Design review of the part built by this model. Coordinates are the model's own, in mm. Face numbers are marked on the shaded views. A direction names the side the tool comes from. Give positions to 0.01 mm unless a question says otherwise; leave off trailing zeros. Loops run counter-clockwise (first coordinate to the right, second up) from the corner with the lowest first, then second, coordinate; pieces in that order, holes last. Notation, with made-up numbers: (-6.75, 78) - (39.25, 78) arc R30 cw to (39.25, 101) - close; hole circle Ø6 at (31.25, 6.5). An arc over 180 degrees is marked (long way). Write each question's results on one line, items separated by ' | '.
from build123d import *

# Parameters (mm, degrees)
SUPPORT_BLOCK_BODY_DEPTH    = 62
CENTRE_START                = 32
CENTRE_CHANNEL_SKETCH_W     = 60
CENTRE_CHANNEL_SKETCH_H     = 88
CENTRE_CHANNEL_CUT_DEPTH    = 124
V_NOTCH_CUT_DEPTH           = 124
BASE_GROOVE_CUT_18X36_REACH = 97.121
FRONT_NOTCH_CUT_REACH       = 159.899
FRONT_NOTCH_SKETCH_W        = 36
FRONT_NOTCH_SKETCH_H        = 12


with BuildPart() as part:
    # Block Profile Sketch → Support Block Body (new, symmetric)
    with BuildSketch(Plane.XY):
        Polygon((-50, 0), (50, 0), (50, 32), (-10, 84), (-50, 84), align=None)
    extrude(amount=SUPPORT_BLOCK_BODY_DEPTH, both=True)

    # Centre Channel Sketch → Centre Channel Cut (cut)
    with BuildSketch(Plane(origin=(0, 0, 0), x_dir=(1, 0, 0), z_dir=(0, 1, 0)).offset(CENTRE_START)):
        with Locations((20, 0)):
            Rectangle(CENTRE_CHANNEL_SKETCH_W, CENTRE_CHANNEL_SKETCH_H)
    extrude(amount=CENTRE_CHANNEL_CUT_DEPTH, mode=Mode.SUBTRACT)

    # V-Notch Sketch → V-Notch Cut (cut)
    with BuildSketch(Plane(origin=(-10, 0, 0), x_dir=(0, 0, -1), z_dir=(1, 0, 0))):
        Polygon((30, 84), (0, 54), (-30, 84), align=None)
    extrude(amount=-V_NOTCH_CUT_DEPTH, mode=Mode.SUBTRACT)

    # Base Groove Sketch → Base Groove Cut 18x36 (cut, up to next)
    with BuildSketch(Plane(origin=(0, 32, 0), x_dir=(1, 0, 0), z_dir=(0, 1, 0)), mode=Mode.PRIVATE) as base_groove_cut_18x36_sk1:
        Polygon((50, 18), (32, 0), (50, -18), align=None)
    base_groove_cut_18x36_tool1 = extrude(base_groove_cut_18x36_sk1.sketch, amount=-BASE_GROOVE_CUT_18X36_REACH, mode=Mode.PRIVATE) & part.part
    add(base_groove_cut_18x36_tool1.solids().sort_by_distance((44, 32, 0))[0], mode=Mode.SUBTRACT)

    # Front Notch Sketch → Front Notch Cut (cut, up to next)
    with BuildSketch(Plane.XY.offset(62), mode=Mode.PRIVATE) as front_notch_cut_sk1:
        with Locations((0, 6)):
            Rectangle(FRONT_NOTCH_SKETCH_W, FRONT_NOTCH_SKETCH_H)
    front_notch_cut_tool1 = extrude(front_notch_cut_sk1.sketch, amount=-FRONT_NOTCH_CUT_REACH, mode=Mode.PRIVATE) & part.part
    add(front_notch_cut_tool1.solids().sort_by_distance((0, 6, 62))[0], mode=Mode.SUBTRACT)


solid = part.part
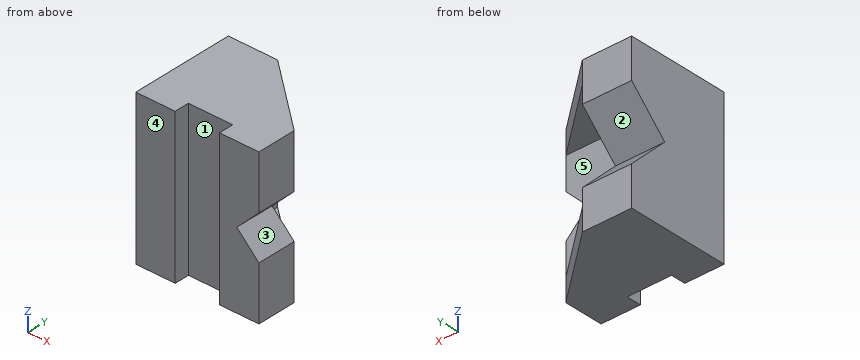
(1) Take a section at D-D on x = -37. Give the boundary of the cut face in (y, z), plus the area to 3 significant figures.
Answers below:
outline: (0, -62) - (84, -62) - (84, -30) - (54, 0) - (84, 30) - (84, 62) - (0, 62) - close | area: 9,520 mm2
(2) Wall thickness on line 1 along X through (y, z) = (8.5, -45); line 2 along Z through (x, y) = (-7.5, 69.5); line 3 along Y through (x, z) = (20, 38.5): over which ranges is each line inside the solid? List them lowest first. Write a range as from..to.
Answers below:
line 1: -50..-18, 18..50 | line 2: -62..-44, 44..62 | line 3: 0..32
(3) Take a section at A-A on x = 41. Give the boundary of the cut face in (y, z).
Answers below:
outline: (0, -62) - (39.8, -62) - (39.8, -44) - (32, -44) - (32, -9) - (0, -9) - close; (0, 9) - (32, 9) - (32, 44) - (39.8, 44) - (39.8, 62) - (0, 62) - close
(4) Take a section at C-C on y = 59.5. Give the boundary of the cut face in (x, z), plus the area to 3 significant figures.
Answers below:
outline: (-50, -62) - (18.27, -62) - (18.27, -44) - (-10, -44) - (-10, -5.5) - (-50, -5.5) - close; (-50, 5.5) - (-10, 5.5) - (-10, 44) - (18.27, 44) - (18.27, 62) - (-50, 62) - close | area: 5,540 mm2
(5) Tool access review of the marked faces 1, 2, 3, 4 and 5: name each direction out of +Z, -Z, +X, -X, +Y, -Y from which nothing blocks a thin tool from reaching the whole face with its end or side.
Answers below:
face 1: +Z, -Z, -Y | face 2: +X, -X, +Y | face 3: +X, +Y, -Y | face 4: +Z, -Z, +X, -X, -Y | face 5: +X, +Y
(6) Take a section at B-B on z = -11. Give the boundary of the cut face in (x, y), plus the area to 3 significant figures.
Answers below:
outline: (-50, 0) - (-18, 0) - (-18, 12) - (18, 12) - (18, 0) - (43, 0) - (43, 32) - (-10, 32) - (-10, 65) - (-50, 65) - close | area: 3,860 mm2
(7) Insertion check: P1, Ø3.5, axis at y = 9, z = 9.5, coming from the +X side; P2, Ø18, axis at x = 6.5, z = -12, coming from the -Y side; P3, Ø18, axis at x = 18, z = 4, coming from the +Y side. Each pin has a flat end and moves straight along its axis. Give the tip position at first contact, or say it passes through.
Answers below:
P1: x = 43.25 | P2: y = 12 | P3: y = 32
